Geometry check sheet. Reference: the model listing, model coordinates, mm. Face numbers are marked on the shaded views. A direction names the side the tool comes from. Give positions to 0.01 mm unless a question says otherwise; leave off trailing zeros. Write each loop counter-clockwise with the first axis right and the second up, starting at its lowest first coordinate (ties: lowest second). Pieces come first, ordered by that corner, then holes.
(1) Cross-section at D-D (y = -49.5). Record the boundary of the cut face in (x, z), and give its area (3 significant figures).
(2) Depth check by flat-ended pin: P1, Ø5, axis at x = 502, y = -8, coming from the -Z side; P2, Ø6, axis at y = 31.5, z = -23, coming from the -X side; P3, Ø3, axis at x = 1072, y = 13, coming from the -Z side. Enter the tip coordinate at first touch or a pass-through.
(3) Cross-section at B-B (x = 342.5). Record the boundary of the cut face in (y, z), and give its area (3 significant figures).
(4) Tool access check on the marked faces 1, 2 and 3. Record the directions out of +Z, -Z, +X, -X, +Y, -Y that give a thin tool (end or side, any length) a straight path to the whole face; none if there is none.
(5) Thickness scan on line 1 along Z through (x, y) = (208, -2.5); line 2 along X through (y, z) = (-47, 35.5); line 3 along Y through (x, z) = (669, -4.5). Record the ranges inside material, lowest first.
(6) Cross-section at C-C (z = 44.5). Record the boundary of the cut face in (x, y), and give its area (3 significant figures).
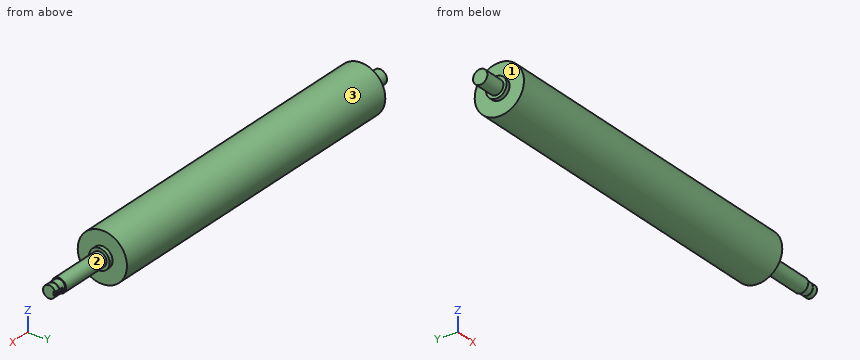
```python
from build123d import *

# Parameters (mm, degrees)
CUT_EXTRUDE_1_DEPTH = 4
SKETCH_3_R          = 15
SKETCH_3_R_2        = 14.3
CUT_EXTRUDE_2_DEPTH = 1.3


with BuildPart() as part:
    # 草图1 → 旋转1 (revolve)
    with BuildSketch(Plane.XY, mode=Mode.PRIVATE) as revolve_1_sk:
        Polygon((0, 0), (0, 17.5), (53, 17.5), (53, 25), (63, 25), (63, 60), (913, 60), (913, 25), (923, 25), (923, 17.5), (1056, 17.5), (1056, 15), (1088, 15), (1088, 0), align=None)
    revolve(revolve_1_sk.sketch.rotate(Axis((1088, 0, 0), (-1, 0, 0)), 90), axis=Axis((1088, 0, 0), (-1, 0, 0)))

    # 草图2 → 切除-拉伸1 (cut)
    with BuildSketch(Plane(origin=(0, 15, 0), x_dir=(1, 0, 0), z_dir=(0, 1, 0))):
        with BuildLine():
            Line((1066, 4), (1098, 4))
            Line((1098, 4), (1098, -4))
            Line((1098, -4), (1066, -4))
            ThreePointArc((1066, -4), (1062, 0), (1066, 4))
        make_face()
    extrude(amount=-CUT_EXTRUDE_1_DEPTH, mode=Mode.SUBTRACT)

    # 草图3 → 切除-拉伸2 (cut)
    with BuildSketch(Plane(origin=(1075.2, 0, 0), x_dir=(0, 0, -1), z_dir=(1, 0, 0))):
        Circle(SKETCH_3_R)
        Circle(SKETCH_3_R_2, mode=Mode.SUBTRACT)
    extrude(amount=-CUT_EXTRUDE_2_DEPTH, mode=Mode.SUBTRACT)


solid = part.part
```
Reply:
1. outline: (63, -33.91) - (913, -33.91) - (913, 33.91) - (63, 33.91) - close
1. area: 57,600 mm2
2. P1: stops at z = -59.75
2. P2: stops at x = 63
2. P3: stops at z = -9.63
3. outline: circle Ø120 at (0, 0)
3. area: 11,300 mm2
4. face 1: -X
4. face 2: +X
4. face 3: +X, -X
5. line 1: z = -59.95 to 59.95
5. line 2: x = 63 to 913
5. line 3: y = -59.83 to 59.83
6. outline: (63, -40.25) - (913, -40.25) - (913, 40.25) - (63, 40.25) - close
6. area: 68,400 mm2
